```python
from build123d import *

# Parameters (mm, degrees)
BASE_PLATE_SKETCH_R        = 1
BASE_PLATE_DEPTH           = 1
UPRIGHT_WALL_SKETCH_W      = 8
UPRIGHT_WALL_SKETCH_H      = 1
UPRIGHT_WALL_DEPTH         = 5
SLOT_CUTS_DEPTH            = 9.246211251
SIDE_LUG_DEPTH             = 0.5
PIN_BOSS_SKETCH_R          = 1.5
PIN_BOSS_SKETCH_R_2        = 0.75
PIN_BOSS_3_DEPTH           = 1
PIN_BORE_SKETCH_R          = 0.75
PIN_BORE_DEPTH             = 8.90569415
UPRIGHT_WALL_FILLET_R1_5_R = 1.5


with BuildPart() as part:
    # Base Plate Sketch → Base Plate (new body)
    with BuildSketch(Plane.XY):
        with BuildLine():
            Line((-2, 2.5), (2, 2.5))
            ThreePointArc((2, 2.5), (3.414213562, 1.914213562), (4, 0.5))
            Line((4, 0.5), (4, -2.5))
            Line((4, -2.5), (-4, -2.5))
            Line((-4, -2.5), (-4, 0.5))
            ThreePointArc((-4, 0.5), (-3.414213562, 1.914213562), (-2, 2.5))
        make_face()
        with Locations((-2, 0.5)):
            Circle(BASE_PLATE_SKETCH_R, mode=Mode.SUBTRACT)
        with Locations((2, 0.5)):
            Circle(BASE_PLATE_SKETCH_R, mode=Mode.SUBTRACT)
    extrude(amount=BASE_PLATE_DEPTH)

    # Upright Wall Sketch → Upright Wall (add)
    with BuildSketch(Plane.XY.offset(1)):
        with Locations((0, -2)):
            Rectangle(UPRIGHT_WALL_SKETCH_W, UPRIGHT_WALL_SKETCH_H)
    extrude(amount=UPRIGHT_WALL_DEPTH)

    # Slot Cuts Sketch → Slot Cuts (cut, through all)
    with BuildSketch(Plane(origin=(0, -1.5, 0), x_dir=(1, 0, 0), z_dir=(0, 1, 0))):
        with BuildLine():
            Line((-4, -2), (-2.8, -2))
            ThreePointArc((-2.8, -2), (-2.234314575, -2.234314575), (-2, -2.8))
            Line((-2, -2.8), (-2, -3.2))
            ThreePointArc((-2, -3.2), (-2.234314575, -3.765685425), (-2.8, -4))
            Line((-2.8, -4), (-4, -4))
            Line((-4, -4), (-4, -2))
        make_face()
        with BuildLine():
            Line((4, -2), (2.8, -2))
            ThreePointArc((2.8, -2), (2.234314575, -2.234314575), (2, -2.8))
            Line((2, -2.8), (2, -3.2))
            ThreePointArc((2, -3.2), (2.234314575, -3.765685425), (2.8, -4))
            Line((2.8, -4), (4, -4))
            Line((4, -4), (4, -2))
        make_face()
    extrude(amount=-SLOT_CUTS_DEPTH, mode=Mode.SUBTRACT)

    # Side Lug Sketch → Side Lug (add, symmetric)
    with BuildSketch(Plane(origin=(0, 0, 0), x_dir=(0, 0, -1), z_dir=(1, 0, 0))):
        with BuildLine():
            Line((-1, 2.5), (-4.5, 2.5))
            ThreePointArc((-4.5, 2.5), (-5.560660172, 2.060660172), (-6, 1))
            Line((-6, 1), (-6, -1.5))
            Line((-6, -1.5), (-1, -1.5))
            Line((-1, -1.5), (-1, 2.5))
        make_face()
    extrude(amount=SIDE_LUG_DEPTH, both=True)

    # Pin Boss Sketch → Pin Boss Ø3 (add, symmetric)
    with BuildSketch(Plane(origin=(0, 0, 0), x_dir=(0, 0, -1), z_dir=(1, 0, 0))):
        with Locations((-4.5, 1)):
            Circle(PIN_BOSS_SKETCH_R)
        with Locations((-4.5, 1)):
            Circle(PIN_BOSS_SKETCH_R_2, mode=Mode.SUBTRACT)
    extrude(amount=PIN_BOSS_3_DEPTH, both=True)

    # Pin Bore Sketch → Pin Bore (cut, through all)
    with BuildSketch(Plane(origin=(0.5, 0, 0), x_dir=(0, 0, -1), z_dir=(1, 0, 0))):
        with Locations((-4.5, 1)):
            Circle(PIN_BORE_SKETCH_R)
    extrude(amount=-PIN_BORE_DEPTH, mode=Mode.SUBTRACT)

    # Upright Wall Fillet R1.5
    upright_wall_fillet_r1_5_edges = [part.edges().sort_by_distance(p)[0] for p in [
        (-4, -2, 6),
        (4, -2, 6),
    ]]
    fillet(upright_wall_fillet_r1_5_edges, radius=UPRIGHT_WALL_FILLET_R1_5_R)


solid = part.part
```
Verification items for the finished model (mm, model axes). A direction names the side the tool comes from. Coordinates: 2 decimals unless noted, no trailing zeros. Loops run counter-clockwise (first coordinate to the right, second up) from the corner with the lowest first, then second, coordinate; pieces in that order, holes last. Notation, with made-up numbers: (7.5, -38.75) - (26.5, -38.75) arc R23 ccw to (26.5, -4.75) - close; hole circle Ø10 at (-39, 21). An arc over 180 degrees is marked (long way). Answer as a JSON object with one key per item and string values.
(1) Cross-section at A-A, the plane x = 0. Record the boundary of the cut face in (y, z).
Response:
{"outline": "(-2.5, 0) - (2.5, 0) - (2.5, 4.5) arc R1.5 ccw to (1, 6) - (-2.5, 6) - close; hole circle Ø1.5 at (1, 4.5)"}
(2) Mould release check, pull along Y, two halves, no side actions. Record for faces 1 (the cylindrical face through (0.01, 2.01, 5.61)), 2 (the cylindrical face through (-3.43, 1.9, 0.49)), 3 (the cylindrical face through (-3.55, -1.99, 5.57)): pulls with the +Y half, pulls with the -Y half, needs draft (parallel to the pull), parting line crosses it, or undercut.
Response:
{"face 1": "undercut", "face 2": "pulls with the +Y half", "face 3": "needs draft"}
(3) Scan lines: line 1 along Y through (x, z) = (0, 4.5); line 2 along Y through (x, z) = (-0.75, 4.5); line 3 along Z through (x, y) = (-0.6, 1). Record each from-to range of solid material in increasing order.
Response:
{"line 1": "y = -2.5 to 0.25, 1.75 to 2.5", "line 2": "y = -2.5 to -1.5, -0.5 to 0.25, 1.75 to 2.5", "line 3": "z = 0 to 1, 3 to 3.75, 5.25 to 6"}
(4) Cross-section at C-C, the plane x = -3.5. Record the boundary of the cut face in (y, z).
Response:
{"outline": "(-2.5, 0) - (1.82, 0) - (1.82, 1) - (-1.5, 1) - (-1.5, 2) - (-2.5, 2) - close; (-2.5, 4) - (-1.5, 4) - (-1.5, 5.62) - (-2.5, 5.62) - close"}
(5) Cross-section at B-B, the plane z = 0.6. Record the boundary of the cut face in (x, y), then the cut area to 3 significant figures.
Response:
{"outline": "(-4, -2.5) - (4, -2.5) - (4, 0.5) arc R2 ccw to (2, 2.5) - (-2, 2.5) arc R2 ccw to (-4, 0.5) - close; hole circle Ø2 at (-2, 0.5); hole circle Ø2 at (2, 0.5)", "area": "32.0 mm²"}
(6) Go/stop test with flat-tipped pins: pin 1 Ø1.5 at (x, z) = (3, 5) entering from +Y; pin 2 Ø1.7 at (y, z) = (1, 4.5) entering from +X; pin 3 Ø1.1 at (x, y) = (3.5, -2) entering from +Z; pin 4 Ø3 at (x, y) = (2, 0.5) entering from +Z. Record where each tip stops, or that it passes through.
Response:
{"pin 1": "stops at y = -1.5", "pin 2": "stops at x = 1", "pin 3": "stops at z = 5.93", "pin 4": "stops at z = 6"}
(7) Access from +Z, -Z, +X, -X, +Y, -Y to the whole of each face (thin tool, end or side, straight path). Record for faces 4 (the flat face through (-1, 2, 4)), 5 (the flat face through (-3, -2, 2)), 6 (the flat face through (3.1, 0.1, 1)), 7 (the flat face through (3, -2, 2)), 8 (the flat face through (-0.5, 0, 3)).
Response:
{"face 4": "+Z, -X, +Y", "face 5": "-X, +Y, -Y", "face 6": "+X, +Y", "face 7": "+X, +Y, -Y", "face 8": "-X"}
(8) Cross-section at D-D, the plane z = 2.45. Record the boundary of the cut face in (x, y), then the cut area to 3 significant figures.
Response:
{"outline": "(-2.08, -2.5) - (2.08, -2.5) - (2.08, -1.5) - (0.5, -1.5) - (0.5, 2.5) - (-0.5, 2.5) - (-0.5, -1.5) - (-2.08, -1.5) - close", "area": "8.16 mm²"}
